from build123d import *

# Parameters (mm, degrees)
SKETCH_1_W          = 328
SKETCH_1_H          = 275
EXTRUDE_1_DEPTH     = 2
EXTRUDE_2_DEPTH     = 328
SKETCH_4_RX         = 120
SKETCH_4_RY         = 100
CUT_EXTRUDE_1_DEPTH = 10


with BuildPart() as part:
    # 草图1 → 凸台-拉伸1 (new body)
    with BuildSketch(Plane.XY):
        Rectangle(SKETCH_1_W, SKETCH_1_H)
    extrude(amount=EXTRUDE_1_DEPTH)

    # 草图2 → 凸台-拉伸2 (add)
    with BuildSketch(Plane.ZY.offset(164)):
        Polygon((0, -137.5), (-103.923048454, -197.5), (-102.923048454, -199.232050808), (1, -139.232050808), (2, -138.654700538), (2, -137.5), align=None)
    extrude(amount=-EXTRUDE_2_DEPTH)

    # 草图4 → 切除-拉伸1 (cut)
    with BuildSketch(Plane(origin=(0, -103.125, 59.53924651), x_dir=(1, 0, 0), z_dir=(0, 0.8660254037844398, -0.49999999999999784))):
        with Locations(Location((0, 188.75), (0, 0, 0))):
            Ellipse(SKETCH_4_RX, SKETCH_4_RY)
    extrude(amount=-CUT_EXTRUDE_1_DEPTH, mode=Mode.SUBTRACT)


solid = part.part
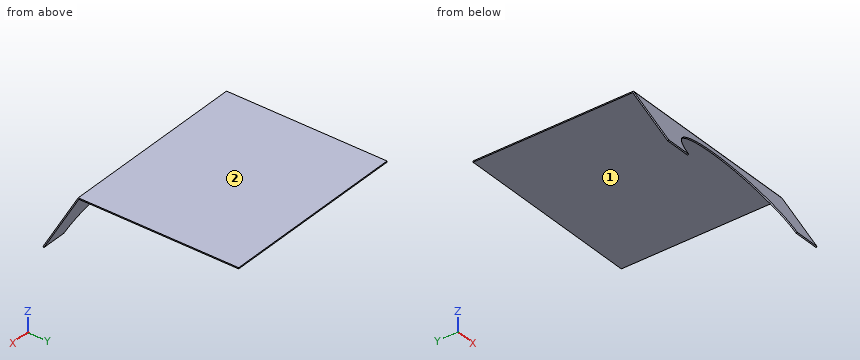
Input: part model. Units: mm. Frame: model coordinates. Face numbers are marked on the shaded views. A direction names the side the tool comes from. Coordinates: 2 decimals unless noted, no trailing zeros. Order: outer loops, then holes, each group sorted by start corner. A loop starts at its lowest first (then second) coordinate and runs counter-clockwise, first axis right, second up. Notation, with made-up numbers: M -24,38.25 L 29,38.25 A31 cw 29,66.25 Z; hole C -2,-40 d10. An arc over 180 degrees is marked long. Write item = value, one per line. Start each with the question number.
(1) First-contact query: P1, Ø6, axis at x = -30, y = 23.5, coming from the -Z side; P2, Ø8, axis at x = -65.5, y = -160.5, coming from the -Z side; P3, Ø8, axis at x = 88.5, y = -154.5, coming from the +Z side. Flat tips, straight axial feed; report the tip coordinate or a pass-through.
(2) Line query: line 1 along Z through (x, y) = (-146.5, 118); line 2 along Y through (x, z) = (-91, -7); line 3 along Y through (x, z) = (-125.5, -10.5). Output: solid intervals per line, ascending. Write a range as [from, to].
(3) Section A-A on y = -31. Output: boundary loops of the cut face in (x, z).
(4) Reachability of the marked faces 1 and 2 from +Z, -Z, +X, -X, +Y, -Y: full face, straight path, thin tool, end or side. Return the list, or none.
(5) Section B-B on z = -12. Output: boundary loops of the cut face in (x, y).
Result set:
q1.P1 = 0
q1.P2 = -32
q1.P3 = -18.52
q2.line_1 = [0, 2]
q2.line_2 = [-143.85, -141.54]
q2.line_3 = [-145.87, -143.56]
q3.outline = M -164,0 L 164,0 L 164,2 L -164,2 Z
q4.face_1 = -Z, +X, -X, +Y
q4.face_2 = +Z, +X, -X, +Y, -Y
q5.outline = M -164,-146.74 L 164,-146.74 L 164,-144.43 L -164,-144.43 Z
